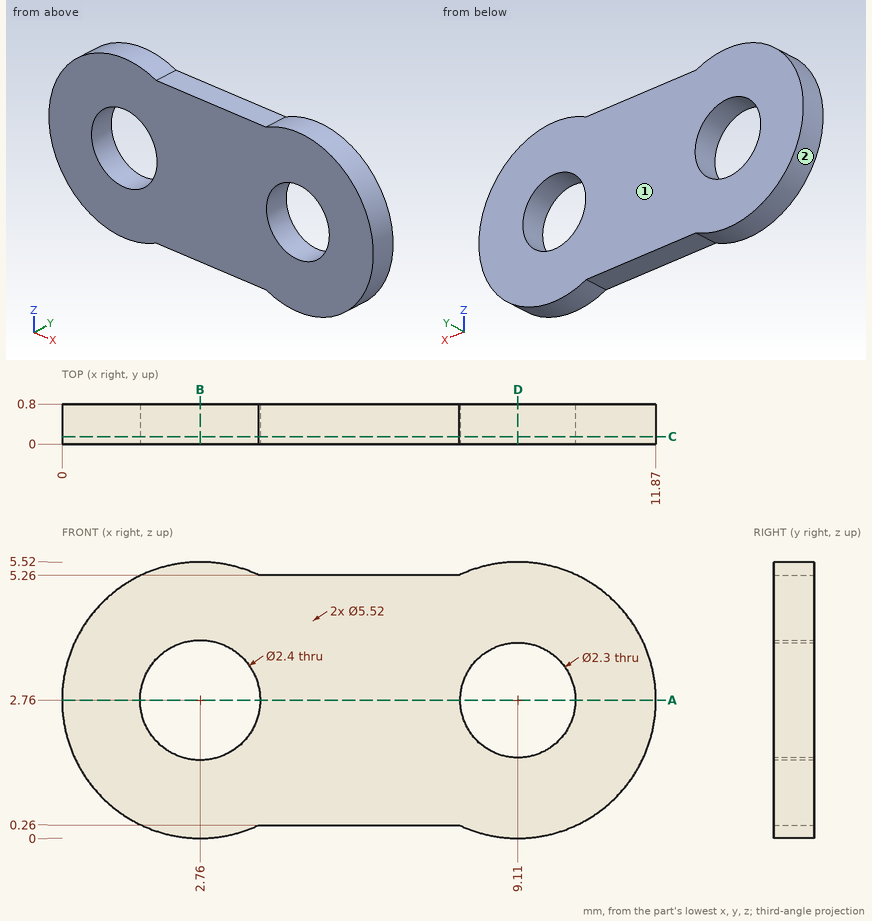
For this review, use the dimensioned drawing (mm, ordinates from the lowest corner) and the shaded views. Round coordinates to 2 decimals unless told otherwise and drop trailing zeros. Write each loop counter-clockwise with the first axis right and the second up, starting at its lowest first coordinate (ties: lowest second). Pieces come first, ordered by that corner, then holes. Notation, with made-up numbers: M -13.5,85.5 L 13.5,85.5 A33 cw 13.5,115.5 Z; hole C -22.5,-28 d2. An arc over 180 degrees is marked long. Use CSV: the item, a comma, the result in double quotes. Start each with the question number.
(1) We need section A-A, the plane z = 2.76. State the section outline as (x, y) points.
(2) Clearance check with flat-ended pins moving along their axes: P1, Ø3, axis at x = 10, z = 2, coming from the -Y side; P2, Ø2, axis at x = 2.76, z = 2.76, coming from the -Y side. State where each tip first meets the part, or that it passes through.
(3) The part is to be moulded in two halves that separate along X. For the marked faces 1 and 2, say which applies: +X half, -X half, draft (parallel to the pull), parting line (faces both ways), or undercut.
(4) We need section D-D, the plane x = 9.11. State the section outline as (y, z) points, then the cut area to 3 significant figures.
(5) We need section C-C, the plane y = 0.15. State the section outline as (x, z) points.
(6) We need section B-B, the plane x = 2.76. State the section outline as (y, z) points, then the cut area to 3 significant figures.
(7) For line 1 along X through (y, z) = (0.25, 2.8); line 2 along Z through (x, y) = (9.5, 0.6); line 3 along Z through (x, y) = (8.75, 0.15), list the stretches that pass through material, from the lowest coordinate up.
Findings:
1,outline,"M 0,0 L 1.56,0 L 1.56,0.8 L 0,0.8 Z; M 3.96,0 L 7.96,0 L 7.96,0.8 L 3.96,0.8 Z; M 10.26,0 L 11.87,0 L 11.87,0.8 L 10.26,0.8 Z"
2,P1,"y = 0"
2,P2,"through"
3,face 1,"draft"
3,face 2,"undercut"
4,outline,"M 0,0 L 0.8,0 L 0.8,1.61 L 0,1.61 Z; M 0,3.91 L 0.8,3.91 L 0.8,5.52 L 0,5.52 Z"
4,area,"2.58 mm^2"
5,outline,"M 3.93,0.26 L 7.94,0.26 A2.76 ccw long 7.94,5.26 L 3.93,5.26 A2.76 ccw long Z; hole C 2.76,2.76 d2.4; hole C 9.11,2.76 d2.3"
6,outline,"M 0,0 L 0.8,0 L 0.8,1.56 L 0,1.56 Z; M 0,3.96 L 0.8,3.96 L 0.8,5.52 L 0,5.52 Z"
6,area,"2.50 mm^2"
7,line 1,"0 to 1.56, 3.96 to 7.96, 10.26 to 11.87"
7,line 2,"0.03 to 1.68, 3.84 to 5.49"
7,line 3,"0.02 to 1.67, 3.85 to 5.5"
